Source: CAD feature listing. Evaluate the final solid. Frame: model axes, mm. A direction names the side the tool comes from. Coordinates: 2 decimals unless noted, no trailing zeros. Order: outer loops, then holes, each group sorted by start corner. A loop starts at its lowest first (then second) coordinate and runs counter-clockwise, first axis right, second up. Notation, with made-up numbers: (30.5, 88) -> (62.5, 88) arc R4 ccw to (62.5, 93) -> close; hole circle Ø3 at (21, 13.25). An arc over 180 degrees is marked (long way). Put each result on its own line as item: value.
from build123d import *

# Parameters (mm, degrees)
BOSS_EXTRUDE1_DEPTH = 1
BOSS_EXTRUDE2_DEPTH = 3
FILLET1_R           = 1.4
SKETCH3_R           = 1.426316434
BOSS_EXTRUDE3_DEPTH = 4.5


with BuildPart() as part:
    # Sketch1 → Boss-Extrude1 (new body)
    with BuildSketch(Plane(origin=(0, 0, 0), x_dir=(1, 0, 0), z_dir=(0, 1, 0))):
        with BuildLine():
            Line((-15, -25.462186482), (-13.267949192, -24.462186482))
            Line((-13.267949192, -24.462186482), (13.267949192, -24.462186482))
            Line((13.267949192, -24.462186482), (15, -25.462186482))
            ThreePointArc((15, -25.462186482), (22.071067812, -22.533254294), (25, -15.462186482))
            Line((25, -15.462186482), (24, -13.730135674))
            Line((24, -13.730135674), (24, 13.730135674))
            Line((24, 13.730135674), (25, 15.462186482))
            ThreePointArc((25, 15.462186482), (22.071067812, 22.533254294), (15, 25.462186482))
            Line((15, 25.462186482), (13.267949192, 24.462186482))
            Line((13.267949192, 24.462186482), (-13.267949192, 24.462186482))
            Line((-13.267949192, 24.462186482), (-15, 25.462186482))
            ThreePointArc((-15, 25.462186482), (-22.071067812, 22.533254294), (-25, 15.462186482))
            Line((-25, 15.462186482), (-24, 13.730135674))
            Line((-24, 13.730135674), (-24, -13.730135674))
            Line((-24, -13.730135674), (-25, -15.462186482))
            ThreePointArc((-25, -15.462186482), (-22.071067812, -22.533254294), (-15, -25.462186482))
        make_face()
    extrude(amount=BOSS_EXTRUDE1_DEPTH)

    # Sketch2 → Boss-Extrude2 (add)
    with BuildSketch(Plane(origin=(0, 1, 0), x_dir=(1, 0, 0), z_dir=(0, 1, 0))):
        Polygon((0, -10.429037626), (7.374443227, -7.374443227), (10.429037626, 0), (-10.429037626, 0), (-7.374443227, -7.374443227), align=None)
        Polygon((0, 10.429037626), (-7.374443227, 7.374443227), (-10.429037626, 0), (10.429037626, 0), (7.374443227, 7.374443227), align=None)
    extrude(amount=BOSS_EXTRUDE2_DEPTH)

    # Fillet1
    fillet1_edges = [part.edges().sort_by_distance(p)[0] for p in [
        (3.687221613, 4, 8.901740426),
        (8.901740426, 4, 3.687221613),
        (8.901740426, 4, -3.687221613),
        (3.687221613, 4, -8.901740426),
        (-3.687221613, 4, -8.901740426),
        (-8.901740426, 4, -3.687221613),
        (-8.901740426, 4, 3.687221613),
        (-3.687221613, 4, 8.901740426),
    ]]
    fillet(fillet1_edges, radius=FILLET1_R)

    # Sketch3 → Boss-Extrude3 (add, symmetric)
    with BuildSketch(Plane.XY):
        with BuildLine():
            ThreePointArc((4, 8.569064594), (0.167778924, 12.565544324), (-3.985925116, 8.904327129))
            Line((-3.985925116, 8.904327129), (-3.985925116, 4))
            Line((-3.985925116, 4), (4, 4))
            Line((4, 4), (4, 8.569064594))
        make_face()
        with Locations((0, 8.569064594)):
            Circle(SKETCH3_R, mode=Mode.SUBTRACT)
    extrude(amount=BOSS_EXTRUDE3_DEPTH, both=True)


solid = part.part
1. Cut plane B-B on x = -12.5. Output: boundary loops of the cut face in (y, z).
Numbers:
outline: (0, -24.46) -> (1, -24.46) -> (1, 24.46) -> (0, 24.46) -> close
2. Set-up query: faces 1 (the flat face through (4, 6, 0)), 2 (the flat face through (1, 7, -4.5)), 3 (the flat face through (-3.986, 6, 0)), 4 (the flat face through (-3.64, 1.79, -8.92)). Return all of +Z, -Z, +X, -X, +Y, -Y with unobstructed straight access to the full face (end or side cutting, diameter ignored); none if empty.
Numbers:
face 1: +Z, -Z, +X, +Y
face 2: -Z, +X, -X, +Y
face 3: +Z, -Z, -X, +Y
face 4: -Z, -X, +Y
3. Cut plane A-A on z = -13. Output: boundary loops of the cut face in (x, y).
Numbers:
outline: (-24, 0) -> (24, 0) -> (24, 1) -> (-24, 1) -> close
4. First-contact query: pin 1 (6.5 mm diameter, centred on x = 1, y = 10, fed in from +Z); pin 2 (5 mm diameter, centred on x = -11, z = -19.5, fed in from +Y); pin 3 (0.5 mm diameter, centred on x = 6.5, y = 0.5, fed in from -Z). Flat tips, straight axial feed; report the tip coordinate or a pass-through.
Numbers:
pin 1: stops at z = 4.5
pin 2: stops at y = 1
pin 3: stops at z = -24.46
5. Pull-direction query (Z, two-part tool) for faces 5 (the flat face through (-8.88, 1.79, -3.74)), 6 (the flat face through (-6, 4, 0)), 7 (the flat face through (8.88, 1.79, 3.74)); classes: pulls with the +Z half, pulls with the -Z half, needs draft (parallel to the pull), parting line crosses it, or undercut.
Numbers:
face 5: pulls with the -Z half
face 6: needs draft
face 7: pulls with the +Z half
6. Ray query, line 1 along Y through (x, z) = (0, -2); line 2 along Z through (x, y) = (-2.5, 8.25); line 3 along Y through (x, z) = (-18.5, -1.5). Return the intervals inside material, ascending.
Numbers:
line 1: y = 0 to 7.14, 10 to 12.57
line 2: z = -4.5 to 4.5
line 3: y = 0 to 1
